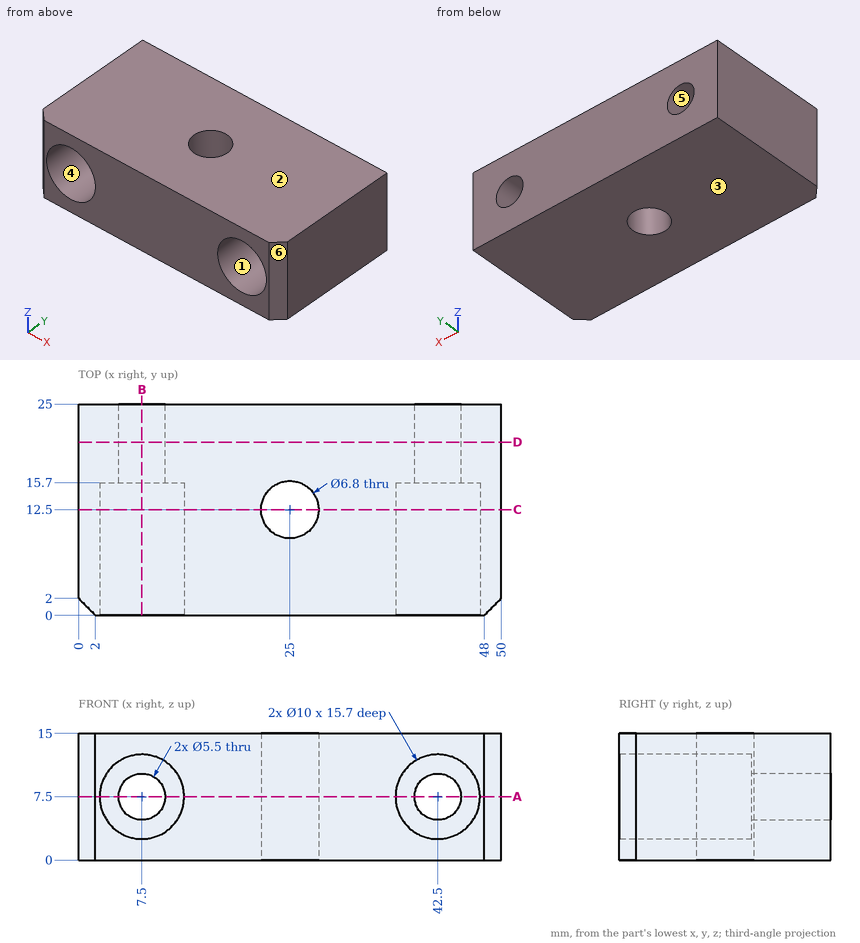
The drawing under review shows one solid part. Ordinate dimensions are in mm from its lowest x, y, z. A direction names the side the tool comes from. Give positions to 0.01 mm unless a question says otherwise; leave off trailing zeros. Order: outer loops, then holes, each group sorted by start corner. A loop starts at its lowest first (then second) coordinate and runs counter-clockwise, first axis right, second up. Notation, with made-up numbers: (86.25, -19) -> (135.25, -19) arc R13 ccw to (135.25, -2) -> close; hole circle Ø3 at (-38, -24.5). An arc over 180 degrees is marked (long way). Write item = value, one per line. Start each with the question number.
(1) We need section C-C on y = 12.5. Write out the cut boundary in (x, z), plus the area to 3 significant figures.
(2) We need section A-A on z = 7.5. Write out the cut boundary in (x, y).
(3) Mouldability with a two-part tool opening along X and no side actions: class the marked faces 3, 4, 5 and 6 as +X half, -X half, draft (parallel to the pull), parting line (faces both ways), or undercut.
(4) We need section B-B on x = 7.5. Write out the cut boundary in (y, z), plus the area to 3 significant figures.
(5) To check wall thickness, follow line 1 along X through (y, z) = (8.5, 10.25); line 2 along Z through (x, y) = (42.5, 5); line 3 along X through (y, z) = (23.75, 9). State the ranges of each line that lie inside material, in increasing order.
(6) For the marked faces 1 and 2, list the 3-axis set-ups (+Z, -Z, +X, -X, +Y, -Y) from which the entire face can be reached by the end or side of a thin tool; tool diameter is ignored.
(7) For pin 1 (6 mm diameter, centred on x = 12.5, y = 5, fed in from -Z); pin 2 (3 mm diameter, centred on x = 43.5, z = 8.5, fed in from -Y), all flat-tipped, find the tip position at first contact; note any pin that passes through.
(8) We need section D-D on y = 20.5. Write out the cut boundary in (x, z), plus the area to 3 significant figures.
Numbers:
q1.outline = (0, 0) -> (21.6, 0) -> (21.6, 15) -> (0, 15) -> close; (28.4, 0) -> (50, 0) -> (50, 15) -> (28.4, 15) -> close; hole circle Ø10 at (7.5, 7.5); hole circle Ø10 at (42.5, 7.5)
q1.area = 491 mm^2
q2.outline = (0, 2) -> (2, 0) -> (2.5, 0) -> (2.5, 15.7) -> (4.75, 15.7) -> (4.75, 25) -> (0, 25) -> close; (10.25, 15.7) -> (12.5, 15.7) -> (12.5, 0) -> (37.5, 0) -> (37.5, 15.7) -> (39.75, 15.7) -> (39.75, 25) -> (10.25, 25) -> close; (45.25, 15.7) -> (47.5, 15.7) -> (47.5, 0) -> (48, 0) -> (50, 2) -> (50, 25) -> (45.25, 25) -> close; hole circle Ø6.8 at (25, 12.5)
q3.face_3 = draft
q3.face_4 = undercut
q3.face_5 = undercut
q3.face_6 = +X half
q4.outline = (0, 0) -> (25, 0) -> (25, 4.75) -> (15.7, 4.75) -> (15.7, 2.5) -> (0, 2.5) -> close; (0, 12.5) -> (15.7, 12.5) -> (15.7, 10.25) -> (25, 10.25) -> (25, 15) -> (0, 15) -> close
q4.area = 167 mm^2
q5.line_1 = 0 to 3.32, 11.68 to 38.32, 46.68 to 50
q5.line_2 = 0 to 2.5, 12.5 to 15
q5.line_3 = 0 to 5.2, 9.8 to 40.2, 44.8 to 50
q6.face_1 = -Y
q6.face_2 = +Z, +X, -X, +Y, -Y
q7.pin_1 = 0
q7.pin_2 = 15.7
q8.outline = (0, 0) -> (50, 0) -> (50, 15) -> (0, 15) -> close; hole circle Ø5.5 at (7.5, 7.5); hole circle Ø5.5 at (42.5, 7.5)
q8.area = 702 mm^2
